Check sheet for the modelled part. Datum: model origin and axes. Units: mm. Give positions to 0.01 mm unless a question says otherwise; leave off trailing zeros. Order: outer loops, then holes, each group sorted by start corner. A loop starts at its lowest first (then second) coordinate and runs counter-clockwise, first axis right, second up.
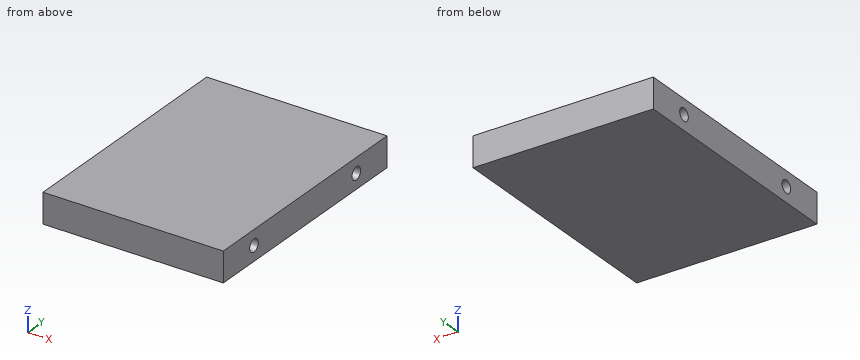
```python
from build123d import *

# Parameters (mm, degrees)
SKETCH_1_W             = 60
SKETCH_1_H             = 80
EXTRUDE_1_DEPTH        = 10
HOLE_WIZARD_M5_1_D     = 4.2
HOLE_WIZARD_M5_1_DEPTH = 14
HOLE_WIZARD_M5_1_TIP   = 1.2618073
HOLE_WIZARD_M5_2_D     = 4.2
HOLE_WIZARD_M5_2_DEPTH = 14
HOLE_WIZARD_M5_2_TIP   = 1.2618073


with BuildPart() as part:
    # 草图1 → 凸台-拉伸1 (new body)
    with BuildSketch(Plane.XY):
        Rectangle(SKETCH_1_W, SKETCH_1_H)
    extrude(amount=EXTRUDE_1_DEPTH)

    # M5 螺纹孔1
    with Locations(Plane(origin=(30, 0, 0), x_dir=(0, 0, -1), z_dir=(1, 0, 0))):
        with Locations((-5, -25), (-5, 25)):
            Hole(HOLE_WIZARD_M5_1_D / 2, depth=HOLE_WIZARD_M5_1_DEPTH)
            with Locations((0, 0, -(HOLE_WIZARD_M5_1_DEPTH + HOLE_WIZARD_M5_1_TIP / 2))):  # 118° drill point
                Cone(0, HOLE_WIZARD_M5_1_D / 2, HOLE_WIZARD_M5_1_TIP, mode=Mode.SUBTRACT)

    # M5 螺纹孔2
    with Locations(Plane.ZY.offset(30)):
        with Locations((5, 25), (5, -25)):
            Hole(HOLE_WIZARD_M5_2_D / 2, depth=HOLE_WIZARD_M5_2_DEPTH)
            with Locations((0, 0, -(HOLE_WIZARD_M5_2_DEPTH + HOLE_WIZARD_M5_2_TIP / 2))):  # 118° drill point
                Cone(0, HOLE_WIZARD_M5_2_D / 2, HOLE_WIZARD_M5_2_TIP, mode=Mode.SUBTRACT)


solid = part.part
```
Q1. Go/stop test with flat-tipped pins: P1, Ø3.5, axis at y = 25, z = 5, coming from the +X side; P2, Ø3.5, axis at y = -25, z = 5, coming from the -X side. Record where each tip stops, or that it passes through.
Q2. Material ranges on line 1 (Y direction, x = 25, z = 5); line 2 (Y direction, x = 18.5, z = 3.25); line 3 (Z direction, x = -27, y = 25), recorded low to high.
Q3. Sectioned sample at A-A, the plane x = -18. Record the cut outline in (y, z), plus the area to 3 significant figures.
Filled in:
1. P1: stops at x = 15.79
1. P2: stops at x = -15.79
2. line 1: y = -40 to -27.1, -22.9 to 22.9, 27.1 to 40
2. line 2: y = -40 to -26.16, -23.84 to 23.84, 26.16 to 40
2. line 3: z = 0 to 2.9, 7.1 to 10
3. outline: (-40, 0) - (40, 0) - (40, 10) - (-40, 10) - close; hole circle Ø4.2 at (-25, 5); hole circle Ø4.2 at (25, 5)
3. area: 772 mm2
